Work out the finished part from the listing and answer in its coordinate system (mm). Face numbers are marked on the shaded views. A direction names the side the tool comes from. Round coordinates to 2 decimals unless told otherwise and drop trailing zeros. Write each loop counter-clockwise with the first axis right and the second up, starting at its lowest first coordinate (ties: lowest second). Pieces come first, ordered by that corner, then holes. Notation, with made-up numbers: (-28.75, -19) - (8.25, -19) arc R24 ccw to (8.25, 12) - close; hole circle Ø9 at (-25, 79.25). An arc over 180 degrees is marked (long way). Answer as a JSON object with one key per item and string values.
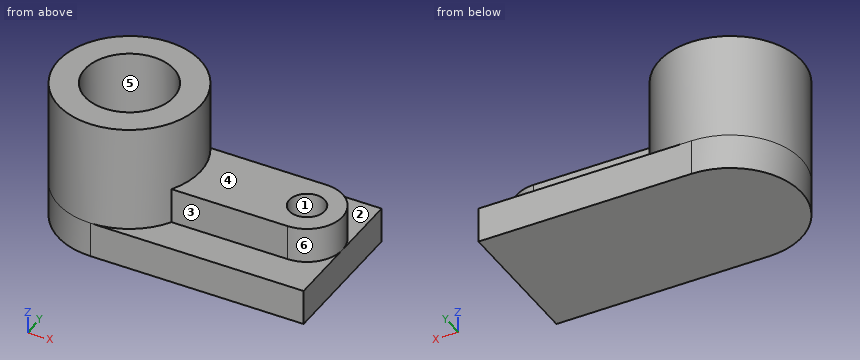
```python
from build123d import *

# Parameters (mm, degrees)
BASE_PLATE_SKETCH_W                = 60
BASE_PLATE_SKETCH_H                = 40
BASE_PLATE_DEPTH                   = 10
CYLINDER_BOSS_SKETCH_40_R          = 20
CYLINDER_BOSS_40_DEPTH             = 40
CYLINDER_ROOT_BOSS_SKETCH_40_R     = 20
CYLINDER_ROOT_BOSS_40_DEPTH        = 10
CYLINDER_START                     = -10
CYLINDER_CLEARANCE_CUT_SKETCH_40_R = 20
CYLINDER_CLEARANCE_CUT_40_DEPTH    = 10
LUG_ARM_DEPTH                      = 10
LUG_HOLE_SKETCH_10_R               = 5
LUG_HOLE_10_DEPTH                  = 10
BORE_SKETCH_25_R                   = 12.5
BORE_25_DEPTH                      = 30


with BuildPart() as part:
    # Base Plate Sketch → Base Plate (new body)
    with BuildSketch(Plane.XY):
        with Locations((30, -20)):
            Rectangle(BASE_PLATE_SKETCH_W, BASE_PLATE_SKETCH_H)
    extrude(amount=BASE_PLATE_DEPTH)

    # Cylinder Boss Sketch Ø40 → Cylinder Boss Ø40 (add)
    with BuildSketch(Plane.XY.offset(10)):
        with Locations(Location((0, -20, 0), (0, 0, 270))):
            Circle(CYLINDER_BOSS_SKETCH_40_R)
    extrude(amount=CYLINDER_BOSS_40_DEPTH)

    # Cylinder Root Boss Sketch Ø40 → Cylinder Root Boss Ø40 (add)
    with BuildSketch(Plane(origin=(0, 0, 0), x_dir=(-1, 0, 0), z_dir=(0, 0, -1))):
        with Locations(Location((0, -20, 0), (0, 0, 90))):
            Circle(CYLINDER_ROOT_BOSS_SKETCH_40_R)
    extrude(amount=-CYLINDER_ROOT_BOSS_40_DEPTH)

    # Cylinder Clearance Cut Sketch Ø40 → Cylinder Clearance Cut Ø40 (cut)
    with BuildSketch(Plane.XY.offset(50).offset(CYLINDER_START)):
        with Locations(Location((0, -20, 0), (0, 0, 90))):
            Circle(CYLINDER_CLEARANCE_CUT_SKETCH_40_R)
    extrude(amount=CYLINDER_CLEARANCE_CUT_40_DEPTH, mode=Mode.SUBTRACT)

    # Lug Arm Sketch → Lug Arm (add)
    with BuildSketch(Plane.XY.offset(10)):
        with BuildLine():
            Line((50, -10), (17.320508076, -10))
            ThreePointArc((17.320508076, -10), (20, -20), (17.320508076, -30))
            Line((17.320508076, -30), (50, -30))
            ThreePointArc((50, -30), (60, -20), (50, -10))
        make_face()
    extrude(amount=LUG_ARM_DEPTH)

    # Lug Hole Sketch Ø10 → Lug Hole Ø10 (cut)
    with BuildSketch(Plane.XY.offset(20)):
        with Locations((50, -20)):
            Circle(LUG_HOLE_SKETCH_10_R)
    extrude(amount=-LUG_HOLE_10_DEPTH, mode=Mode.SUBTRACT)

    # Bore Sketch Ø25 → Bore Ø25 (cut)
    with BuildSketch(Plane.XY.offset(40)):
        with Locations((0, -20)):
            Circle(BORE_SKETCH_25_R)
    extrude(amount=-BORE_25_DEPTH, mode=Mode.SUBTRACT)


solid = part.part
```
Item 1: A cutting plane is placed at D-D (z = 8). Write down the section's boundary in (x, y).
Results found:
{"outline": "(0, -40) - (60, -40) - (60, 0) - (0, 0) arc R20 ccw to start"}
Item 2: For the marked faces 1, 2 and 3, determine the directions among +Z, -Z, +X, -X, +Y, -Y from which every point of the face is accessible in a straight line to the end or side of a thin tool.
Results found:
{"face 1": "+Z", "face 2": "+Z, +X, +Y", "face 3": "+Z, +X, -Y"}
Item 3: Consider line 1 along Y through (x, z) = (0, 17.5); line 2 along Z through (x, y) = (9.5, -20.5); line 3 along Z through (x, y) = (31, -27). Determine where each line is inside the solid, lowest interval first.
Results found:
{"line 1": "-40 to -32.5, -7.5 to 0", "line 2": "0 to 10", "line 3": "0 to 20"}
Item 4: A cutting plane is placed at B-B (z = 33). Write down the section's boundary in (x, y).
Results found:
{"outline": "circle Ø40 at (0, -20); hole circle Ø25 at (0, -20)"}
Item 5: A cutting plane is placed at C-C (x = -8.5). Write down the section's boundary in (y, z).
Results found:
{"outline": "(-38.1, 0) - (-1.9, 0) - (-1.9, 40) - (-10.83, 40) - (-10.83, 10) - (-29.17, 10) - (-29.17, 40) - (-38.1, 40) - close"}
Item 6: Determine the mould class of the marked faces 4, 5 and 6 for opening direction Y: pulls with the +Y half, pulls with the -Y half, needs draft (parallel to the pull), parting line crosses it, or undercut.
Results found:
{"face 4": "needs draft", "face 5": "undercut", "face 6": "parting line crosses it"}
Item 7: A cutting plane is placed at A-A (y = -36). Write down the section's boundary in (x, z), and give its area (3 significant figures).
Results found:
{"outline": "(-12, 0) - (60, 0) - (60, 10) - (12, 10) - (12, 40) - (-12, 40) - close", "area": "1,440 mm²"}
Item 8: Each of these flat-tipped pins is pushed along its axis until it touches: P1, Ø3, axis at x = -9, z = 34.5, coming from the -Y side; P2, Ø6, axis at x = 5.5, z = 21.5, coming from the +Y side; P3, Ø8, axis at x = 40.5, z = 17, coming from the -Y side. Where does it stop, or does it pass through?
Results found:
{"P1": "y = -38.54", "P2": "y = -0.16", "P3": "y = -30"}
